Verification items for the finished model (mm, model axes). Face numbers are marked on the shaded views. A direction names the side the tool comes from. Round coordinates to 2 decimals unless told otherwise and drop trailing zeros. Order: outer loops, then holes, each group sorted by start corner. A loop starts at its lowest first (then second) coordinate and runs counter-clockwise, first axis right, second up. Notation, with made-up numbers: (-35.75, -33) -> (-0.75, -33) arc R26 cw to (-0.75, -2) -> close; hole circle Ø8 at (57, 82.25). An arc over 180 degrees is marked (long way). Return JSON: item names as keys, results as strings. Group by question number.
1) Depth check by flat-ended pin: pin 1 (0.6 mm diameter, centred on x = 1, z = -16.5, fed in from +Y); pin 2 (16.5 mm diameter, centred on y = 99, z = -19.5, fed in from -X); pin 3 (1 mm diameter, centred on y = 63, z = -7, fed in from +X); pin 4 (2.5 mm diameter, centred on x = 23.5, y = 90.5, fed in from +Z). Enter the tip coordinate at first touch or a pass-through.
2) Section check C-C on x = 0. Enter the section's corners in (y, z).
3) Tool access check on the marked faces 5, 6 and 7. Record the directions out of +Z, -Z, +X, -X, +Y, -Y that give a thin tool (end or side, any length) a straight path to the whole face; none if there is none.
4) Section check D-D on y = 13.5. Enter the section's corners in (x, z).
5) Draft check along X on the marked faces 1, 2, 3 and 4. Enter one of: pulls with the +X half, pulls with the -X half, needs draft (parallel to the pull), parting line crosses it, or undercut.
6) Section check B-B on y = 78.5. Enter the section's corners in (x, z).
7) Scan lines: L1, parallel to X at y = -1.5, z = 12; L2, parallel to X at y = 97, z = -18; L3, parallel to Z at x = -10.5, y = 102. Record each from-to range of solid material in increasing order.
8) Section check A-A on z = 21.5. Enter the section's corners in (x, y), plus the area to 3 significant figures.
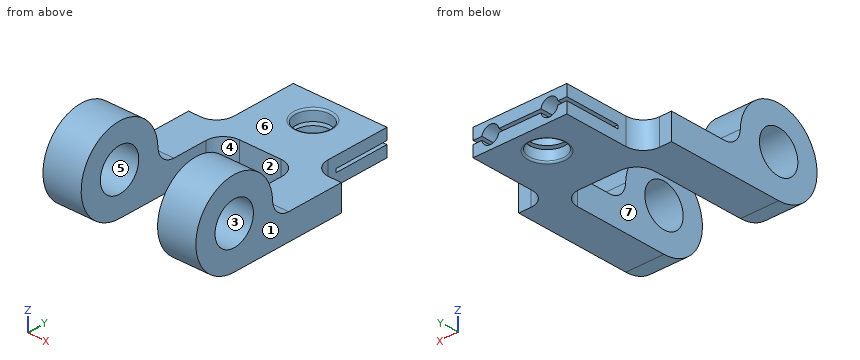
```python
from build123d import *

# Parameters (mm, degrees)
LUG_BARREL_SKETCH_R           = 24.01
LUG_BARREL_SKETCH_R_2         = 12
ROLLER_LUG_BARREL_DEPTH       = 44
MOUNTING_PLATE_DEPTH          = 44
PLATE_TO_BARREL_FILLET_R10_R  = 10
PLATE_SHOULDER_CUT_DEPTH      = 125.533048224
PLATE_SHOULDER_CUT_DEPTH_BACK = 125.533048224
PLATE_SHOULDER_CUT_SKETCH_W   = 44
PLATE_SHOULDER_CUT_SKETCH_H   = 88.01
LUG_GAP_CUT_DEPTH             = 125.533048224
LUG_GAP_CUT_DEPTH_BACK        = 125.533048224
LUG_GAP_SKETCH_W              = 17
LUG_GAP_SKETCH_H              = 47
LUG_GAP_FILLET_R10_R          = 10
CLAMP_SLIT_2MM_DEPTH          = 125.533048224
CLAMP_SLIT_2MM_DEPTH_BACK     = 125.533048224
CLAMP_SLIT_SKETCH_W           = 2
CLAMP_SLIT_SKETCH_H           = 32
PLATE_HOLE_20_DEPTH           = 127.579304786
PLATE_HOLE_20_DEPTH_BACK      = 127.579304786
PLATE_HOLE_SKETCH_R           = 10
PLATE_HOLE_EDGE_FILLET_R1_R   = 1
CLAMP_SCREW_SKETCH_R          = 5
CLAMP_SCREW_CUT_DEPTH         = 49


with BuildPart() as part:
    # Lug Barrel Sketch → Roller Lug Barrel (new, symmetric)
    with BuildSketch(Plane(origin=(0, 0, 0), x_dir=(0, 0, -1), z_dir=(1, 0, 0))):
        Circle(LUG_BARREL_SKETCH_R)
        Circle(LUG_BARREL_SKETCH_R_2, mode=Mode.SUBTRACT)
    extrude(amount=ROLLER_LUG_BARREL_DEPTH, both=True)

    # Mounting Plate Sketch → Mounting Plate (add, symmetric)
    with BuildSketch(Plane(origin=(0, 0, 0), x_dir=(0, 0, -1), z_dir=(1, 0, 0))):
        with BuildLine():
            Line((24.01, 0), (24.01, 114))
            Line((24.01, 114), (9.01, 114))
            Line((9.01, 114), (9.01, 22.255336439))
            ThreePointArc((9.01, 22.255336439), (19.909924661, 13.419202659), (24.01, 0))
        make_face()
    extrude(amount=MOUNTING_PLATE_DEPTH, both=True)

    # Plate to Barrel Fillet R10
    plate_to_barrel_fillet_r10_edges = [part.edges().sort_by_distance(p)[0] for p in [
        (0, 22.255336439, -9.01),
    ]]
    fillet(plate_to_barrel_fillet_r10_edges, radius=PLATE_TO_BARREL_FILLET_R10_R)

    # Plate Shoulder Cut Sketch → Plate Shoulder Cut (cut, two sides: drawn at the far end of the back side and taken through both)
    with BuildSketch(Plane.XY.offset(-PLATE_SHOULDER_CUT_DEPTH_BACK)):
        with Locations((0, 19.995)):
            Rectangle(PLATE_SHOULDER_CUT_SKETCH_W, PLATE_SHOULDER_CUT_SKETCH_H)
    extrude(amount=PLATE_SHOULDER_CUT_DEPTH + PLATE_SHOULDER_CUT_DEPTH_BACK, mode=Mode.SUBTRACT)

    # Lug Gap Sketch → Lug Gap Cut (cut, two sides: drawn at the far end of the back side and taken through both)
    with BuildSketch(Plane.XY.offset(-LUG_GAP_CUT_DEPTH_BACK)):
        with Locations((-35.5, 90.5)):
            Rectangle(LUG_GAP_SKETCH_W, LUG_GAP_SKETCH_H)
        with Locations((35.5, 90.5)):
            Rectangle(LUG_GAP_SKETCH_W, LUG_GAP_SKETCH_H)
    extrude(amount=LUG_GAP_CUT_DEPTH + LUG_GAP_CUT_DEPTH_BACK, mode=Mode.SUBTRACT)

    # Lug Gap Fillet R10
    lug_gap_fillet_r10_edges = [part.edges().sort_by_distance(p)[0] for p in [
        (-22, 64, -16.51),
        (22, 64, -16.51),
        (-27, 67, -16.51),
        (27, 67, -16.51),
    ]]
    fillet(lug_gap_fillet_r10_edges, radius=LUG_GAP_FILLET_R10_R)

    # Clamp Slit Sketch → Clamp Slit 2mm (cut, two sides: drawn at the far end of the back side and taken through both)
    with BuildSketch(Plane(origin=(0, 0, 0), x_dir=(0, 0, -1), z_dir=(1, 0, 0)).offset(-CLAMP_SLIT_2MM_DEPTH_BACK)):
        with Locations((16.51, 98)):
            Rectangle(CLAMP_SLIT_SKETCH_W, CLAMP_SLIT_SKETCH_H)
    extrude(amount=CLAMP_SLIT_2MM_DEPTH + CLAMP_SLIT_2MM_DEPTH_BACK, mode=Mode.SUBTRACT)

    # Plate Hole Sketch → Plate Hole Ø20 (cut, two sides: drawn at the far end of the back side and taken through both)
    with BuildSketch(Plane.XY.offset(-9.01).offset(-PLATE_HOLE_20_DEPTH_BACK)):
        with Locations((0, 97)):
            Circle(PLATE_HOLE_SKETCH_R)
    extrude(amount=PLATE_HOLE_20_DEPTH + PLATE_HOLE_20_DEPTH_BACK, mode=Mode.SUBTRACT)

    # Plate Hole Edge Fillet R1
    plate_hole_edge_fillet_r1_edges = [part.edges().sort_by_distance(p)[0] for p in [
        (-10, 97, -9.01),
        (-10, 97, -24.01),
    ]]
    fillet(plate_hole_edge_fillet_r1_edges, radius=PLATE_HOLE_EDGE_FILLET_R1_R)

    # Clamp Screw Sketch → Clamp Screw Cut (cut)
    with BuildSketch(Plane(origin=(0, 114, 0), x_dir=(1, 0, 0), z_dir=(0, 1, 0))):
        with Locations(Location((-17, 16.51, 0), (0, 0, 270))):
            Circle(CLAMP_SCREW_SKETCH_R)
        with Locations(Location((17, 16.51, 0), (0, 0, 270))):
            Circle(CLAMP_SCREW_SKETCH_R)
    extrude(amount=-CLAMP_SCREW_CUT_DEPTH, mode=Mode.SUBTRACT)


solid = part.part
```
Check result:
{
 "1": {"pin 1": "y = 82", "pin 2": "x = -27", "pin 3": "through", "pin 4": "z = -9.01"},
 "2": {"outline": "(64, -24.01) -> (86, -24.01) arc R1 ccw to (87, -23.01) -> (87, -17.51) -> (82, -17.51) -> (82, -15.51) -> (87, -15.51) -> (87, -10.01) arc R1 ccw to (86, -9.01) -> (64, -9.01) -> close; (107, -23.01) arc R1 ccw to (108, -24.01) -> (114, -24.01) -> (114, -17.51) -> (107, -17.51) -> close; (107, -15.51) -> (114, -15.51) -> (114, -9.01) -> (108, -9.01) arc R1 ccw to (107, -10.01) -> close"},
 "3": {"face 5": "+X, -X", "face 6": "+Z, +X, -X, +Y", "face 7": "+Z, -Z, -Y"},
 "4": {"outline": "(-44, -24.01) -> (-22, -24.01) -> (-22, 19.86) -> (-44, 19.86) -> close; (22, -24.01) -> (44, -24.01) -> (44, 19.86) -> (22, 19.86) -> close"},
 "5": {"face 1": "pulls with the +X half", "face 2": "undercut", "face 3": "needs draft", "face 4": "undercut"},
 "6": {"outline": "(-27, -24.01) -> (27, -24.01) -> (27, -9.01) -> (-27, -9.01) -> close; hole circle Ø10 at (-17, -16.51); hole circle Ø10 at (17, -16.51)"},
 "7": {"L1": "-44 to -22, 22 to 44", "L2": "-27 to -21.77, -12.23 to -10, 10 to 12.23, 21.77 to 27", "L3": "-24.01 to -17.51, -15.51 to -9.01"},
 "8": {"outline": "(-44, -10.69) -> (-22, -10.69) -> (-22, 10.69) -> (-44, 10.69) -> close; (22, -10.69) -> (44, -10.69) -> (44, 10.69) -> (22, 10.69) -> close", "area": "941 mm^2"}
}
